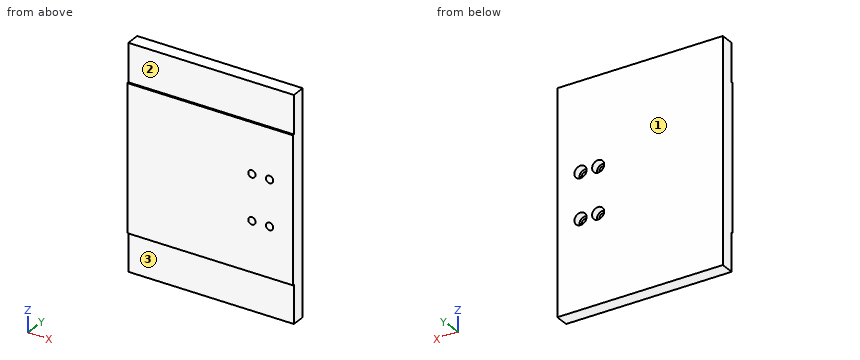
from build123d import *

# Parameters (mm, degrees)
SKETCH_1_W                = 150
SKETCH_1_H                = 200
EXTRUDE_1_DEPTH           = 14
SKETCH_2_W                = 150
SKETCH_2_H                = 34.5
CUT_EXTRUDE_1_DEPTH       = 1.5
HOLE_WIZARD_1_D           = 6.6
HOLE_WIZARD_1_CBORE_D     = 11
HOLE_WIZARD_1_CBORE_DEPTH = 6.8


with BuildPart() as part:
    # 草图1 → 凸台-拉伸1 (new body)
    with BuildSketch(Plane(origin=(0, 0, 0), x_dir=(1, 0, 0), z_dir=(0, 1, 0))):
        Rectangle(SKETCH_1_W, SKETCH_1_H)
    extrude(amount=EXTRUDE_1_DEPTH)

    # 草图2 → 切除-拉伸1 (cut)
    with BuildSketch(Plane.XZ):
        with Locations((0, 82.75)):
            Rectangle(SKETCH_2_W, SKETCH_2_H)
        with Locations((0, -82.75)):
            Rectangle(SKETCH_2_W, SKETCH_2_H)
    extrude(amount=-CUT_EXTRUDE_1_DEPTH, mode=Mode.SUBTRACT)

    # 打孔尺寸(%根据)内六角圆柱头螺钉的类型1 (through all)
    with Locations(Plane(origin=(37.95, 14, 20.5), x_dir=(0, 0, 1), z_dir=(0, 1, 0))):
        with Locations((0, 0), (-41, 0), (0, 16), (-41, 16)):
            CounterBoreHole(HOLE_WIZARD_1_D / 2, HOLE_WIZARD_1_CBORE_D / 2, HOLE_WIZARD_1_CBORE_DEPTH)


solid = part.part
Geometry: final body of the model. Coordinates: model frame, mm. Face numbers are marked on the shaded views. A direction names the side the tool comes from. Round coordinates to 2 decimals unless told otherwise and drop trailing zeros. Loops run counter-clockwise (first coordinate to the right, second up) from the corner with the lowest first, then second, coordinate; pieces in that order, holes last. Notation, with made-up numbers: (13, -19.5) -> (62, -19.5) arc R35 ccw to (62, 17.5) -> close; hole circle Ø1 at (71, 4). An arc over 180 degrees is marked (long way). One line per question, with ' | ' between items. Start each with the question number.
1. Contact query for flat-ended pins moving along their axis: pin 1 (5.5 mm diameter, centred on x = 36.5, z = 21, fed in from +Y); pin 2 (10.5 mm diameter, centred on x = 10.5, z = 84.5, fed in from -Y); pin 3 (0.8 mm diameter, centred on x = 31, y = 1, fed in from -Z). Output: stop coordinate, or through.
2. Line query: line 1 along X through (y, z) = (10, 20.5); line 2 along X through (y, z) = (3, -20.5); line 3 along Z through (x, y) = (36, 9.5). Output: solid intervals per line, ascending. Write a range as [from, to].
3. Section C-C on x = -12.5. Output: boundary loops of the cut face in (y, z).
4. Section B-B on z = -20.5. Output: boundary loops of the cut face in (x, y), and give its area (3 significant figures).
5. Section A-A on x = 37.95. Output: boundary loops of the cut face in (y, z), and give its area (3 significant figures).
6. Set-up query: the marked faces 1, 2 and 3. Return all of +Z, -Z, +X, -X, +Y, -Y with unobstructed straight access to the full face (end or side cutting, diameter ignored); none if empty.
7. Section D-D on z = -77. Output: boundary loops of the cut face in (x, y), and give its area (4 significant figures).
Returned:
1) pin 1: stops at y = 7.2 | pin 2: stops at y = 1.5 | pin 3: stops at z = -65.5
2) line 1: x = [-75, 32.45], [43.45, 48.45], [59.45, 75] | line 2: x = [-75, 34.65], [41.25, 50.65], [57.25, 75] | line 3: z = [-100, -25.64], [-15.36, 15.36], [25.64, 100]
3) outline: (0, -65.5) -> (1.5, -65.5) -> (1.5, -100) -> (14, -100) -> (14, 100) -> (1.5, 100) -> (1.5, 65.5) -> (0, 65.5) -> close
4) outline: (-75, 0) -> (34.65, 0) -> (34.65, 7.2) -> (32.45, 7.2) -> (32.45, 14) -> (-75, 14) -> close; (41.25, 0) -> (50.65, 0) -> (50.65, 7.2) -> (48.45, 7.2) -> (48.45, 14) -> (43.45, 14) -> (43.45, 7.2) -> (41.25, 7.2) -> close; (57.25, 0) -> (75, 0) -> (75, 14) -> (59.45, 14) -> (59.45, 7.2) -> (57.25, 7.2) -> close | area: 1,860 mm2
5) outline: (0, -65.5) -> (1.5, -65.5) -> (1.5, -100) -> (14, -100) -> (14, -26) -> (7.2, -26) -> (7.2, -23.8) -> (0, -23.8) -> close; (0, -17.2) -> (7.2, -17.2) -> (7.2, -15) -> (14, -15) -> (14, 15) -> (7.2, 15) -> (7.2, 17.2) -> (0, 17.2) -> close; (0, 23.8) -> (7.2, 23.8) -> (7.2, 26) -> (14, 26) -> (14, 100) -> (1.5, 100) -> (1.5, 65.5) -> (0, 65.5) -> close | area: 2,450 mm2
6) face 1: +Z, -Z, +X, -X, +Y | face 2: +Z, +X, -X, -Y | face 3: -Z, +X, -X, -Y
7) outline: (-75, 1.5) -> (75, 1.5) -> (75, 14) -> (-75, 14) -> close | area: 1,875 mm2
